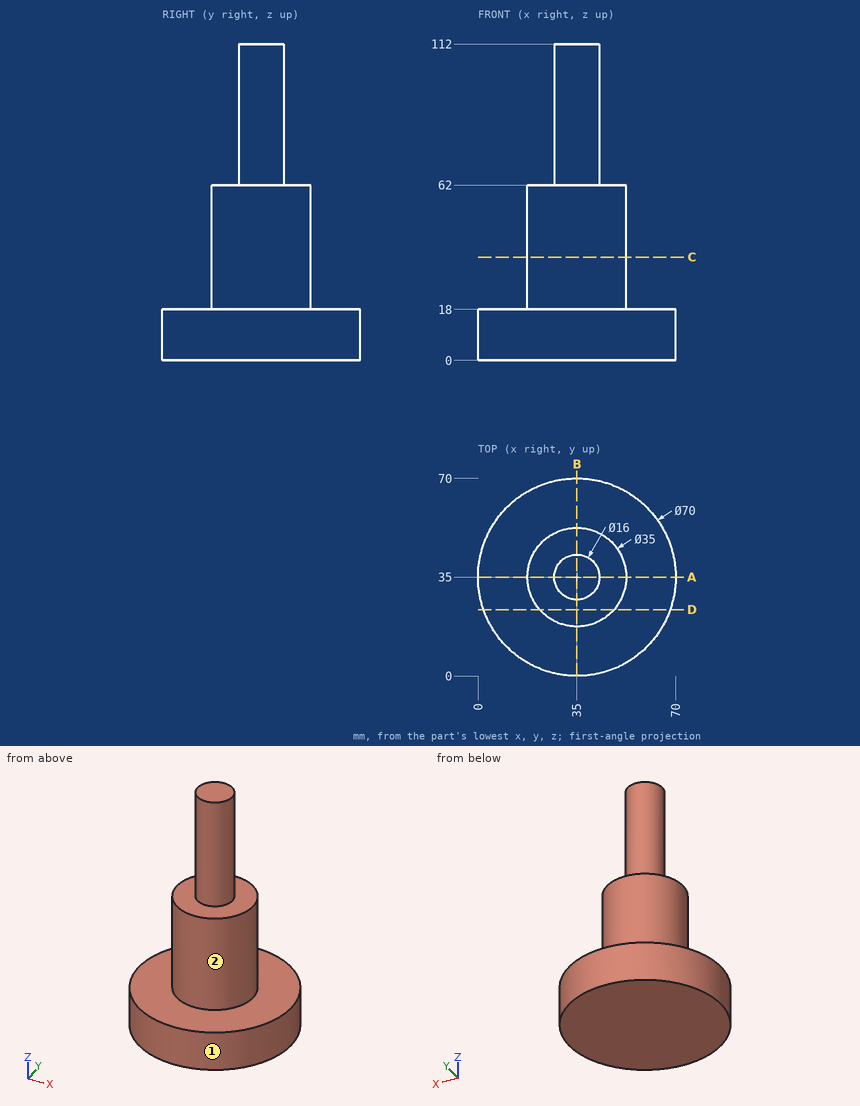
The drawing under review shows one solid part. Ordinate dimensions are in mm from its lowest x, y, z. A direction names the side the tool comes from. Round coordinates to 2 decimals unless told otherwise and drop trailing zeros. Loops run counter-clockwise (first coordinate to the right, second up) from the corner with the lowest first, then second, coordinate; pieces in that order, holes last.
Item 1: For line 1 (Z direction, x = 35.5, y = 50); line 2 (Z direction, x = 16, y = 36); line 3 (Y direction, x = 49.5, z = 16), list the stretches that pass through material, from the lowest coordinate up.
Determined:
line 1: z = 0 to 62
line 2: z = 0 to 18
line 3: y = 3.14 to 66.86
Item 2: Take a section at C-C (z = 36.5). Write out the cut boundary in (x, y), then the cut area to 3 significant figures.
Determined:
outline: circle Ø35 at (35, 35)
area: 962 mm2
Item 3: Clearance check with flat-ended pins moving along their axes: pin 1 Ø3 at (x, y) = (33.5, 46) entering from -Z; pin 2 Ø5 at (x, z) = (30, 29.5) entering from +Y; pin 3 Ø5 at (x, z) = (51, 40) entering from +Y; pin 4 Ø10 at (x, z) = (22.5, 28) entering from +Y. State where each tip first meets the part, or that it passes through.
Determined:
pin 1: stops at z = 0
pin 2: stops at y = 52.32
pin 3: stops at y = 46.14
pin 4: stops at y = 50.81
Item 4: Take a section at D-D (y = 23.5). Write out the cut boundary in (x, z), then the cut area to 3 significant figures.
Determined:
outline: (1.94, 0) - (68.06, 0) - (68.06, 18) - (48.19, 18) - (48.19, 62) - (21.81, 62) - (21.81, 18) - (1.94, 18) - close
area: 2,350 mm2
Item 5: For the marked faces 1 and 2, list the 3-axis set-ups (+Z, -Z, +X, -X, +Y, -Y) from which the entire face can be reached by the end or side of a thin tool; tool diameter is ignored.
Determined:
face 1: +Z, -Z
face 2: +Z
Item 6: Take a section at A-A (y = 35). Write out the cut boundary in (x, z).
Determined:
outline: (0, 0) - (70, 0) - (70, 18) - (52.5, 18) - (52.5, 62) - (43, 62) - (43, 112) - (27, 112) - (27, 62) - (17.5, 62) - (17.5, 18) - (0, 18) - close
